Input: part model. Units: mm. Frame: model coordinates. A direction names the side the tool comes from. Round coordinates to 2 decimals unless told otherwise and drop trailing zeros. Order: outer loops, then holes, each group sorted by start corner. A loop starts at its lowest first (then second) coordinate and runs counter-clockwise, first axis right, second up.
Item 1: Cut plane B-B on y = 36.5. Output: boundary loops of the cut face in (x, z), then the cut area to 3 significant figures.
Item 2: Reachability of faces 1 (the flat face through (234.379, 13, -5)), 2 (the flat face through (84.379, 17, 5)), 3 (the flat face through (84.379, 28, -5)), 4 (the flat face through (93, 22, -7)), 5 (the cylindrical face through (246, 32, 5)) from +Z, -Z, +X, -X, +Y, -Y: full face, straight path, thin tool, end or side. Return the list, or none.
Item 3: Cut plane C-C on x = 79. Output: boundary loops of the cut face in (y, z), then the cut area to 3 significant figures.
Item 4: Line query: L1, parallel to Z at x = 144.5, y = 22; L2, parallel to X at y = 29, z = 8.5; L3, parallel to Y at x = 177, z = -3. Output: solid intervals per line, ascending.
Item 5: First-contact query: pin 1 (10.5 mm diameter, centred on x = 92.5, z = 3, fed in from -Y); pin 2 (1.5 mm diameter, centred on x = 218.5, z = -9, fed in from -Y); pin 3 (10.5 mm diameter, centred on x = 93, y = 23.5, fed in from +Z); pin 4 (17 mm diameter, centred on y = 24, z = 1.5, fed in from -X). Flat tips, straight axial feed; report the tip coordinate or a pass-through.
Item 6: Mould query, pull axis Z, two halves, no side actions, for faces 6 (the cylindrical face through (235.393, 12.287, -1.302)), 7 (the flat face through (102.379, 22.1, 7.2)), 8 (the conical face through (234.525, 18.012, -0.55)). Classes: released by +Z, released by -Z, zero draft, split by the parting line, or undercut.
Item 7: Cut plane A-A on x = 217. Output: boundary loops of the cut face in (y, z).
```python
from build123d import *

# Parameters (mm, degrees)
SKETCH2_R          = 25.69251773
SKETCH2_W          = 14
SKETCH2_H          = 14
CUT_EXTRUDE1_DEPTH = 18
SKETCH4_R          = 2.5
CUT_EXTRUDE3_DEPTH = 10


with BuildPart() as part:
    # Sketch1 → Revolve1 (revolve)
    with BuildSketch(Plane.XY, mode=Mode.PRIVATE) as revolve1_sk:
        with BuildLine():
            Line((254.379291769, 33.201574447), (254.379291769, 30.851574447))
            Line((254.379291769, 30.851574447), (237.379291769, 30.851574447))
            Line((237.379291769, 30.851574447), (234.379291769, 26.201574447))
            Line((234.379291769, 26.201574447), (172.647910202, 26.201574447))
            Line((172.647910202, 26.201574447), (66.379291769, 26.201574447))
            Line((66.379291769, 26.201574447), (66.379291769, 28.201574447))
            ThreePointArc((66.379291769, 28.201574447), (73.620533102, 32.172747161), (81.379291769, 29.343002876))
            Line((81.379291769, 29.343002876), (81.379291769, 29.201574447))
            Line((81.379291769, 29.201574447), (84.379291769, 29.201574447))
            Line((84.379291769, 29.201574447), (84.379291769, 31.701574447))
            Line((84.379291769, 31.701574447), (102.379291769, 31.701574447))
            Line((102.379291769, 31.701574447), (102.379291769, 32.784579692))
            ThreePointArc((102.379291769, 32.784579692), (115.381258369, 38.170170595), (127.608048324, 31.201574447))
            Line((127.608048324, 31.201574447), (228.379291769, 31.201574447))
            ThreePointArc((228.379291769, 31.201574447), (230.500612112, 32.080254104), (231.379291769, 34.201574447))
            Line((231.379291769, 34.201574447), (234.379291769, 34.201574447))
            Line((234.379291769, 34.201574447), (234.379291769, 32.201574447))
            Line((234.379291769, 32.201574447), (236.379291769, 32.201574447))
            Line((236.379291769, 32.201574447), (236.379291769, 33.201574447))
            Line((236.379291769, 33.201574447), (254.379291769, 33.201574447))
        make_face()
    revolve(revolve1_sk.sketch.rotate(Axis((62.379291769, 22.201574447, 0), (1, 0, 0)), 90), axis=Axis((62.379291769, 22.201574447, 0), (1, 0, 0)))

    # Sketch2 → Cut-Extrude1 (cut)
    with BuildSketch(Plane.ZY.offset(-84.379291769)):
        with Locations((0, 22.201574447)):
            Circle(SKETCH2_R)
        with Locations((0, 22.201574447)):
            Rectangle(SKETCH2_W, SKETCH2_H, mode=Mode.SUBTRACT)
    extrude(amount=-CUT_EXTRUDE1_DEPTH, mode=Mode.SUBTRACT)

    # Sketch4 → Cut-Extrude3 (cut)
    with BuildSketch(Plane(origin=(0, 29.201574447, 0), x_dir=(1, 0, 0), z_dir=(0, 1, 0))):
        with Locations(Location((246.379291769, 0, 0), (0, 0, 90))):
            Circle(SKETCH4_R)
    extrude(amount=CUT_EXTRUDE3_DEPTH, mode=Mode.SUBTRACT)


solid = part.part
```
From the geometry:
1. outline: circle Ø14.36 at (114.38, 0)
1. area: 162 mm2
2. face 1: none
2. face 2: +Z, -Y
2. face 3: -Z, +Y
2. face 4: -Z, +Y, -Y
2. face 5: +X
3. outline: circle Ø17.74 at (22.2, 0); hole circle Ø8 at (22.2, 0)
3. area: 197 mm2
4. L1: z = -9 to -3.99, 3.99 to 9
4. L2: x = 102.65 to 126.11, 231.16 to 234.38, 236.38 to 254.38
4. L3: y = 13.72 to 19.56, 24.85 to 30.69
5. pin 1: stops at y = 15.2
5. pin 2: stops at y = 18.6
5. pin 3: stops at z = 7
5. pin 4: stops at x = 66.38
6. face 6: split by the parting line
6. face 7: zero draft
6. face 8: undercut
7. outline: circle Ø18 at (22.2, 0); hole circle Ø8 at (22.2, 0)
